Could you check a few things on this drawing? It's one solid part, dimensions in mm from its lowest x, y, z. A direction names the side the tool comes from. Coordinates: 2 decimals unless noted, no trailing zeros. Order: outer loops, then holes, each group sorted by start corner. A loop starts at its lowest first (then second) coordinate and runs counter-clockwise, first axis right, second up. Notation, with made-up numbers: M -34,25 L -16,25 A29 ccw -16,63 Z; hole C -22,-12.5 d1. An arc over 180 degrees is marked long. Write item = value, one per line. Start each with the question number.
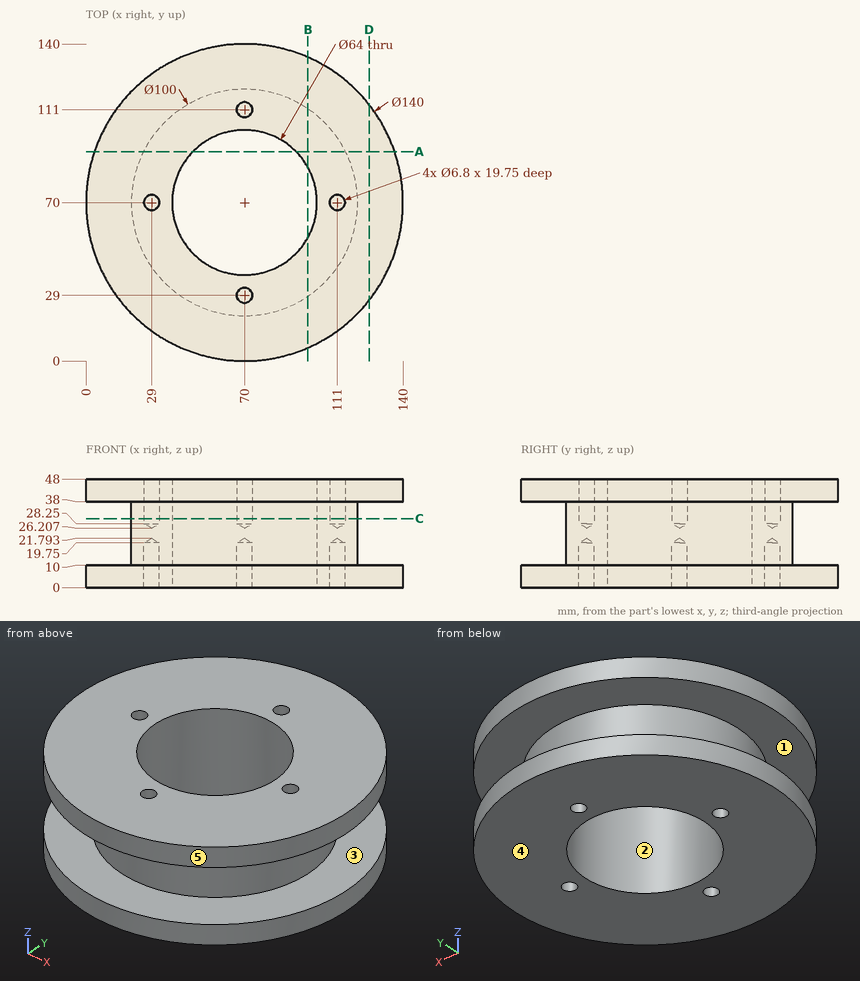
(1) Imagine slicing it at A-A on y = 92.5. List the corners of the cut face in (x, z) for me, plus the area to 3 significant figures.
(2) Imagine slicing it at C-C on z = 30.5. List the corners of the cut face in (x, y) for me.
(3) Please list where these lines run through material, in increasing order: probe 1 along Y at (x, z) = (70, 14); probe 2 along Z at (x, y) = (48, 13.5). Write a range as from..to.
(4) Imagine slicing it at B-B on x = 98. List the corners of the cut face in (y, z) for me, plus the area to 3 significant figures.
(5) For the marked faces 1 and 2, which set-ups out of +Z, -Z, +X, -X, +Y, -Y let a thin tool reach every point of the face, with its end or its side?
(6) Will these pins go through, and if not, where does the flat tip stop? P1, Ø11, axis at x = 70, y = 111, coming from the -Z side; P2, Ø5.5, axis at x = 111, y = 70, coming from the -Z side; P3, Ø2, axis at y = 111, z = 22, coming from the +X side; P4, Ø10, axis at x = 34.5, z = 14, coming from the -Y side.
(7) Thinking about a two-plate mould opening in Z: for the marked faces 3, 4 and 5, which applies, released by +Z, released by -Z, zero draft, split by the parting line, or undercut?
(8) Imagine slicing it at D-D on x = 125. List the corners of the cut face in (y, z) for me.
Response:
q1.outline = M 3.71,0 L 47.25,0 L 47.25,48 L 3.71,48 L 3.71,38 L 25.35,38 L 25.35,10 L 3.71,10 Z; M 92.75,0 L 136.29,0 L 136.29,10 L 114.65,10 L 114.65,38 L 136.29,38 L 136.29,48 L 92.75,48 Z
q1.area = 2,970 mm2
q2.outline = C 70,70 d100; hole C 29,70 d6.8; hole C 70,70 d64; hole C 70,29 d6.8; hole C 70,111 d6.8; hole C 111,70 d6.8
q3.probe_1 = 20..25.6, 32.4..38, 102..107.6, 114.4..120
q3.probe_2 = 0..10, 38..48
q4.outline = M 5.84,0 L 54.51,0 L 54.51,48 L 5.84,48 L 5.84,38 L 28.58,38 L 28.58,10 L 5.84,10 Z; M 85.49,0 L 134.16,0 L 134.16,10 L 111.42,10 L 111.42,38 L 134.16,38 L 134.16,48 L 85.49,48 Z
q4.area = 3,400 mm2
q5.face_1 = none
q5.face_2 = +Z, -Z
q6.P1 = 0
q6.P2 = 20.14
q6.P3 = 100
q6.P4 = 8
q7.face_3 = undercut
q7.face_4 = released by -Z
q7.face_5 = zero draft
q8.outline = M 26.7,0 L 113.3,0 L 113.3,10 L 26.7,10 Z; M 26.7,38 L 113.3,38 L 113.3,48 L 26.7,48 Z
